from build123d import *

# Parameters (mm, degrees)
BOSS_EXTRUDE1_DEPTH         = 7
SKETCH2_R                   = 5.75
BOSS_EXTRUDE2_DEPTH         = 11
SKETCH3_R                   = 2
CUT_EXTRUDE1_DEPTH          = 10
M4_TAPPED_HOLE1_D           = 3.3
M4_TAPPED_HOLE1_CSINK_D     = 4.05
M4_TAPPED_HOLE1_CSINK_ANGLE = 90
SKETCH6_R                   = 1.5
CUT_EXTRUDE2_DEPTH          = 21.199009877


with BuildPart() as part:
    # Sketch1 → Boss-Extrude1 (new body)
    with BuildSketch(Plane(origin=(0, 0, 0), x_dir=(0, 0, -1), z_dir=(1, 0, 0))):
        Polygon((6.92820323, 0), (3.464101615, 6), (-3.464101615, 6), (-6.92820323, 0), (-3.464101615, -6), (3.464101615, -6), align=None)
    extrude(amount=BOSS_EXTRUDE1_DEPTH)

    # Sketch2 → Boss-Extrude2 (add)
    with BuildSketch(Plane(origin=(7, 0, 0), x_dir=(0, 0, -1), z_dir=(1, 0, 0))):
        Circle(SKETCH2_R)
    extrude(amount=BOSS_EXTRUDE2_DEPTH)

    # Sketch3 → Cut-Extrude1 (cut)
    with BuildSketch(Plane(origin=(18, 0, 0), x_dir=(0, 0, -1), z_dir=(1, 0, 0))):
        Circle(SKETCH3_R)
    extrude(amount=-CUT_EXTRUDE1_DEPTH, mode=Mode.SUBTRACT)

    # M4 Tapped Hole1 (through all)
    with Locations(Plane.ZY):
        with Locations((0, 0)):
            CounterSinkHole(M4_TAPPED_HOLE1_D / 2, M4_TAPPED_HOLE1_CSINK_D / 2, counter_sink_angle=M4_TAPPED_HOLE1_CSINK_ANGLE)

    # Sketch6 → Cut-Extrude2 (cut, through all)
    with BuildSketch(Plane(origin=(0, 0, 0), x_dir=(1, 0, 0), z_dir=(0, 1, 0))):
        with Locations(Location((14.8, 0, 0), (0, 0, 270))):
            Circle(SKETCH6_R)
    extrude(amount=-CUT_EXTRUDE2_DEPTH, mode=Mode.SUBTRACT)


solid = part.part
Here's how the part is built. I have some questions about the finished solid (model axes, mm). A direction names the side the tool comes from. Round coordinates to 2 decimals unless told otherwise and drop trailing zeros. Loops run counter-clockwise (first coordinate to the right, second up) from the corner with the lowest first, then second, coordinate; pieces in that order, holes last. Notation, with made-up numbers: M 15.25,-24 L 48.25,-24 A26 ccw 48.25,6 Z; hole C -11.75,-33 d1. An arc over 180 degrees is marked long. Write each question's results on one line, items separated by ' | '. Start each with the question number.
(1) Thinking about a two-plate mould opening in X: for faces 3 (the cylindrical face through (14.225, -3.508, 1.386)), 4 (the cylindrical face through (4.241, 1.115, 1.216)), 5 (the flat face through (18, 0.1, -2.5)), 6 (the flat face through (0, 1, 2)), which applies, pulls with the +X half, pulls with the -X half, needs draft (parallel to the pull), parting line crosses it, or undercut?
(2) I want a section at B-B (z = 0). Please give me the cut outline in (x, y) (3 decimals), then the cut area to 3 significant figures.
(3) I want a section at A-A (x = 6.5). Please give me the cut outline in (y, z), then the cut area to 3 significant figures.
(4) If I drill on probe 1 along Y at (x, z) = (4.75, 0); probe 2 along X at (y, z) = (-2.2, 0); probe 3 along Z at (x, y) = (14.8, -3.85), over which ranges is the centre line in solid material (lowest first)? Write a range as from..to.
(5) I want a section at C-C (y = -2.5). Please give me the cut outline in (x, z), then the cut area to 3 significant figures.
(6) Will these pins go through, and if not, where does the flat tip stop? P1, Ø5, axis at x = 10.5, z = 2, coming from the -Y side; P2, Ø3.5, axis at y = 0, z = 0, coming from the +X side; P3, Ø5, axis at x = 14.8, z = 0, coming from the +Y side.
(7) I want a section at D-D (y = 4). Please give me the cut outline in (x, z), then the cut area to 3 significant figures.
(8) On a 3-axis mill with a long thin cutter (end or side, diameter ignored), from which of +Z, -Z, +X, -X, +Y, -Y can I reach the whole of each face in a straight line? I mean faces 1 (the flat face through (3, 6, 0)), 2 (the cylindrical face through (13, 2, 0)). Say none if no direction works.
Solved:
1) face 3: undercut | face 4: needs draft | face 5: pulls with the +X half | face 6: pulls with the -X half
2) outline: M 0,-6 L 7,-6 L 7,-5.75 L 13.3,-5.75 L 13.3,-2 L 8,-2 L 8,-1.65 L 0.375,-1.65 L 0,-2.025 Z; M 0,2.025 L 0.375,1.65 L 8,1.65 L 8,2 L 18,2 L 18,5.75 L 7,5.75 L 7,6 L 0,6 Z; M 16.3,-5.75 L 18,-5.75 L 18,-2 L 16.3,-2 Z | area: 133 mm²
3) outline: M -6,-3.46 L 0,-6.93 L 6,-3.46 L 6,3.46 L 0,6.93 L -6,3.46 Z; hole C 0,0 d3.3 | area: 116 mm²
4) probe 1: y = -6..-1.65, 1.65..6 | probe 2: x = 0..13.3, 16.3..18 | probe 3: z = -4.27..-1.5, 1.5..4.27
5) outline: M 0,-5.48 L 7,-5.48 L 7,-5.18 L 18,-5.18 L 18,5.18 L 7,5.18 L 7,5.48 L 0,5.48 Z; hole C 14.8,0 d3 | area: 184 mm²
6) P1: stops at y = -5.75 | P2: stops at x = 8 | P3: stops at y = 5.75
7) outline: M 0,-4.62 L 7,-4.62 L 7,-4.13 L 18,-4.13 L 18,4.13 L 7,4.13 L 7,4.62 L 0,4.62 Z | area: 156 mm²
8) face 1: +Z, -Z, +X, -X, +Y | face 2: +X
